Part model, mm, in its own coordinate system. Face numbers are marked on the shaded views. Coordinates: 2 decimals unless noted, no trailing zeros. Loops run counter-clockwise (first coordinate to the right, second up) from the corner with the lowest first, then second, coordinate; pieces in that order, holes last. Notation, with made-up numbers: (26, -23) - (32, -23) arc R15 ccw to (32, -4) - close; hole circle Ø9 at (59.5, 79.25). An arc over 180 degrees is marked (long way). Use a Markdown table: item, result. Add a question column.
1. Wall check: probe 1 along Z at (x, y) = (-52, -15); probe 2 along Z at (x, y) = (47.5, -26); probe 3 along Z at (x, y) = (13, 3.5). Give the ranges that are in metal, low to high. Write a range as [from, to].
2. Band-saw the part on C-C, the plane z = 60. Give the cut face in (x, y).
3. Band-saw the part on B-B, the plane z = 305.5. Give the cut face in (x, y).
4. Drop flat-ended pins along their axis: pin 1 (8 mm diameter, centred on x = 26, z = 244, fed in from +Y); pin 2 (1 mm diameter, centred on x = -23, z = 507, fed in from -Y); pin 3 (4 mm diameter, centred on y = 16.5, z = 402, fed in from -X); pin 4 (5 mm diameter, centred on x = 29, y = 9.5, fed in from -Z). Give the stop position or say it passes through.
5. Band-saw the part on A-A, the plane y = -40. Give the cut face in (x, z).
6. Pull direction Z, two halves, no side cores. Call the marked faces 1, 2 and 3: pulls with the +Z half, pulls with the -Z half, needs draft (parallel to the pull), parting line crosses it, or undercut.
from build123d import *

# Parameters (mm, degrees)
FLANGE_SKETCH_R               = 60
FLANGE_120X16_DEPTH           = 16
FRONT_SHAFT_SKETCH_R          = 25
FRONT_SHAFT_50X62_DEPTH       = 62
CRANK_WEB_1_DEPTH             = 22
CRANKPIN_1_SKETCH_R           = 22.5
CRANKPIN_1_45_DEPTH           = 35
CRANK_WEB_2_DEPTH             = 22
CRANKPIN_2_SKETCH_R           = 22.5
CRANKPIN_2_45_DEPTH           = 35
CRANK_WEB_3_DEPTH             = 22
CENTRE_MAIN_JOURNAL_SKETCH_R  = 25
CENTRE_MAIN_JOURNAL_50_DEPTH  = 45
CRANK_WEB_4_DEPTH             = 22
CRANKPIN_3_SKETCH_R           = 22.5
CRANKPIN_3_45_DEPTH           = 35
CRANK_WEB_5_DEPTH             = 22
CRANKPIN_4_SKETCH_R           = 20
CRANKPIN_4_40_DEPTH           = 35
CRANK_WEB_6_DEPTH             = 22
REAR_SHAFT_SKETCH_R           = 22.5
REAR_SHAFT_45X145_DEPTH       = 145
REAR_START                    = -100
REAR_SHAFT_STEP_SKETCH_R      = 25
REAR_SHAFT_STEP_50X100_DEPTH  = 100
REAR_SHAFT_PROFILE_CUT_DEPTH  = 100
END_STUB_SKETCH_R             = 12.5
END_STUB_25X20_DEPTH          = 20
FLANGE_BOLT_HOLES_SKETCH_R    = 6
FLANGE_BOLT_HOLES_4X_12_DEPTH = 20


with BuildPart() as part:
    # Flange Sketch → Flange Ø120x16 (new body)
    with BuildSketch(Plane.XY):
        Circle(FLANGE_SKETCH_R)
    extrude(amount=FLANGE_120X16_DEPTH)

    # Front Shaft Sketch → Front Shaft Ø50x62 (add)
    with BuildSketch(Plane.XY.offset(16)):
        Circle(FRONT_SHAFT_SKETCH_R)
    extrude(amount=FRONT_SHAFT_50X62_DEPTH)

    # Crank Web 1 Sketch → Crank Web 1 (add)
    with BuildSketch(Plane.XY.offset(78)):
        with BuildLine():
            Line((0, -27.5), (-40, -27.5))
            ThreePointArc((-40, -27.5), (-67.5, 0), (-40, 27.5))
            Line((-40, 27.5), (0, 27.5))
            ThreePointArc((0, 27.5), (27.5, 0), (0, -27.5))
        make_face()
    extrude(amount=CRANK_WEB_1_DEPTH)

    # Crankpin 1 Sketch → Crankpin 1 Ø45 (add)
    with BuildSketch(Plane.XY.offset(100)):
        with Locations((-40, 0)):
            Circle(CRANKPIN_1_SKETCH_R)
    extrude(amount=CRANKPIN_1_45_DEPTH)

    # Crank Web 2 Sketch → Crank Web 2 (add)
    with BuildSketch(Plane.XY.offset(135)):
        with BuildLine():
            Line((-40, 27.5), (40, 27.5))
            ThreePointArc((40, 27.5), (67.5, 0), (40, -27.5))
            Line((40, -27.5), (-40, -27.5))
            ThreePointArc((-40, -27.5), (-67.5, 0), (-40, 27.5))
        make_face()
    extrude(amount=CRANK_WEB_2_DEPTH)

    # Crankpin 2 Sketch → Crankpin 2 Ø45 (add)
    with BuildSketch(Plane.XY.offset(157)):
        with Locations((40, 0)):
            Circle(CRANKPIN_2_SKETCH_R)
    extrude(amount=CRANKPIN_2_45_DEPTH)

    # Crank Web 3 Sketch → Crank Web 3 (add)
    with BuildSketch(Plane.XY.offset(192)):
        with BuildLine():
            Line((40, -27.5), (0, -27.5))
            ThreePointArc((0, -27.5), (-27.5, 0), (0, 27.5))
            Line((0, 27.5), (40, 27.5))
            ThreePointArc((40, 27.5), (67.5, 0), (40, -27.5))
        make_face()
    extrude(amount=CRANK_WEB_3_DEPTH)

    # Centre Main Journal Sketch → Centre Main Journal Ø50 (add)
    with BuildSketch(Plane.XY.offset(214)):
        Circle(CENTRE_MAIN_JOURNAL_SKETCH_R)
    extrude(amount=CENTRE_MAIN_JOURNAL_50_DEPTH)

    # Crank Web 4 Sketch → Crank Web 4 (add)
    with BuildSketch(Plane.XY.offset(259)):
        with BuildLine():
            Line((0, 27.5), (40, 27.5))
            ThreePointArc((40, 27.5), (67.5, 0), (40, -27.5))
            Line((40, -27.5), (0, -27.5))
            ThreePointArc((0, -27.5), (-27.5, 0), (0, 27.5))
        make_face()
    extrude(amount=CRANK_WEB_4_DEPTH)

    # Crankpin 3 Sketch → Crankpin 3 Ø45 (add)
    with BuildSketch(Plane.XY.offset(281)):
        with Locations((40, 0)):
            Circle(CRANKPIN_3_SKETCH_R)
    extrude(amount=CRANKPIN_3_45_DEPTH)

    # Crank Web 5 Sketch → Crank Web 5 (add)
    with BuildSketch(Plane.XY.offset(316)):
        with BuildLine():
            Line((40, -27.5), (-40, -27.5))
            ThreePointArc((-40, -27.5), (-67.5, 0), (-40, 27.5))
            Line((-40, 27.5), (40, 27.5))
            ThreePointArc((40, 27.5), (67.5, 0), (40, -27.5))
        make_face()
    extrude(amount=CRANK_WEB_5_DEPTH)

    # Crankpin 4 Sketch → Crankpin 4 Ø40 (add)
    with BuildSketch(Plane.XY.offset(338)):
        with Locations((-40, 0)):
            Circle(CRANKPIN_4_SKETCH_R)
    extrude(amount=CRANKPIN_4_40_DEPTH)

    # Crank Web 6 Sketch → Crank Web 6 (add)
    with BuildSketch(Plane.XY.offset(373)):
        with BuildLine():
            Line((-40, 27.5), (0, 27.5))
            ThreePointArc((0, 27.5), (27.5, 0), (0, -27.5))
            Line((0, -27.5), (-40, -27.5))
            ThreePointArc((-40, -27.5), (-67.5, 0), (-40, 27.5))
        make_face()
    extrude(amount=CRANK_WEB_6_DEPTH)

    # Rear Shaft Sketch → Rear Shaft Ø45x145 (add)
    with BuildSketch(Plane.XY.offset(395)):
        Circle(REAR_SHAFT_SKETCH_R)
    extrude(amount=REAR_SHAFT_45X145_DEPTH)

    # Rear Shaft Step Sketch → Rear Shaft Step Ø50x100 (add)
    with BuildSketch(Plane.XY.offset(540).offset(REAR_START)):
        Circle(REAR_SHAFT_STEP_SKETCH_R)
    extrude(amount=REAR_SHAFT_STEP_50X100_DEPTH)

    # Rear Shaft Cut Sketch → Rear Shaft Profile Cut (cut)
    with BuildSketch(Plane.XY.offset(540).offset(REAR_START)):
        with BuildLine():
            Line((-24.494897428, -5), (-22.5, -5))
            Line((-22.5, -5), (-22.5, 5))
            Line((-22.5, 5), (-24.494897428, 5))
            ThreePointArc((-24.494897428, 5), (-25, 0), (-24.494897428, -5))
        make_face()
    extrude(amount=REAR_SHAFT_PROFILE_CUT_DEPTH, mode=Mode.SUBTRACT)

    # End Stub Sketch → End Stub Ø25x20 (add)
    with BuildSketch(Plane.XY.offset(540)):
        Circle(END_STUB_SKETCH_R)
    extrude(amount=END_STUB_25X20_DEPTH)

    # Flange Bolt Holes Sketch → Flange Bolt Holes 4xØ12 (cut)
    with BuildSketch(Plane.XY.offset(16)):
        with Locations((0, 40)):
            Circle(FLANGE_BOLT_HOLES_SKETCH_R)
        with Locations((0, -40)):
            Circle(FLANGE_BOLT_HOLES_SKETCH_R)
        with Locations((-40, 0)):
            Circle(FLANGE_BOLT_HOLES_SKETCH_R)
        with Locations((40, 0)):
            Circle(FLANGE_BOLT_HOLES_SKETCH_R)
    extrude(amount=-FLANGE_BOLT_HOLES_4X_12_DEPTH, mode=Mode.SUBTRACT)


solid = part.part
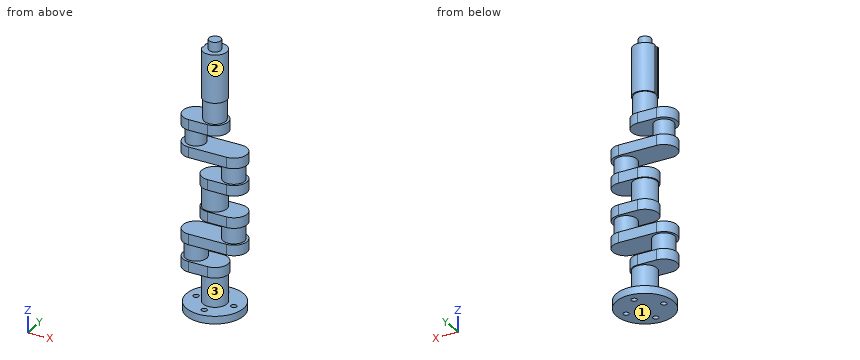
Geometry check:
| question | item | result |
|---|---|---|
| 1 | probe 1 | z = [0, 16], [78, 157], [316, 395] |
| 1 | probe 2 | z = [0, 16], [135, 157], [192, 214], [259, 281], [316, 338] |
| 1 | probe 3 | z = [0, 100], [135, 157], [192, 281], [316, 338], [373, 540] |
| 2 | outline | circle Ø50 at (0, 0) |
| 3 | outline | circle Ø45 at (40, 0) |
| 4 | pin 1 | stops at y = 11.87 |
| 4 | pin 2 | stops at y = -10.9 |
| 4 | pin 3 | stops at x = -17.2 |
| 4 | pin 4 | stops at z = 0 |
| 5 | outline | (-44.72, 0) - (-6, 0) - (-6, 16) - (-44.72, 16) - close; (6, 0) - (44.72, 0) - (44.72, 16) - (6, 16) - close |
| 6 | face 1 | pulls with the -Z half |
| 6 | face 2 | needs draft |
| 6 | face 3 | undercut |
